CAD build for the part. Positions are in the model's coordinates, mm. Face numbers are marked on the shaded views. A direction names the side the tool comes from. Coordinates: 2 decimals unless noted, no trailing zeros. Loops run counter-clockwise (first coordinate to the right, second up) from the corner with the lowest first, then second, coordinate; pieces in that order, holes last.
1) Saw through at B-B, the plane x = 0. Write the cut outline in (y, z).
2) Saw through at D-D, the plane x = -11.5. Write the cut outline in (y, z).
3) Saw through at C-C, the plane z = -4.5. Write the cut outline in (x, y), and give its area (3 significant figures).
4) Pin check, flat tips, straight feed: pin 1 Ø15.5 at (x, z) = (-24, 0) entering from +Y; pin 2 Ø6.5 at (y, z) = (36, -13.5) entering from +X; pin 3 Ø4 at (x, z) = (-14.5, -19.5) entering from +Y. Stop position of each tip, or through.
5) Which spindle directions (+Z, -Z, +X, -X, +Y, -Y) get a long thin tool onto all of the face, cutting with end or side? Do the marked faces 1, 2, 3, 4 and 5. Say none if no direction does.
6) Wall check: line 1 along X through (y, z) = (5, 0); line 2 along X through (y, z) = (60, -19); line 3 along Y through (x, z) = (0, -14). Give the ranges that are in metal, low to high.
7) Two-plate mould, pull along X, no slides. Class the marked faces 6, 7 and 8: +X half, -X half, draft (parallel to the pull), parting line (faces both ways), or undercut.
8) Saw through at A-A, the plane z = -19. Write the cut outline in (x, y).
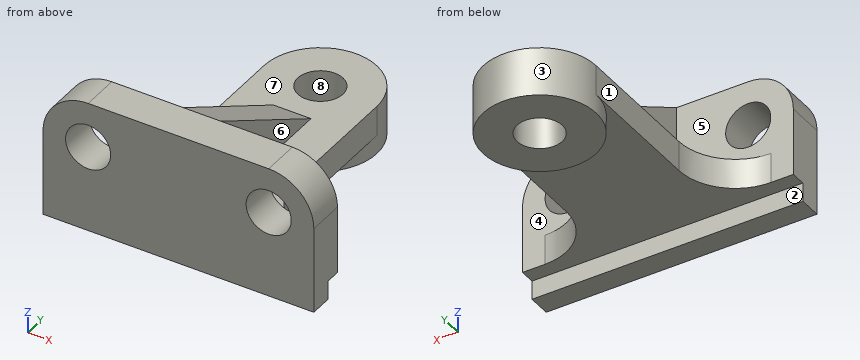
```python
from build123d import *

# Parameters (mm, degrees)
BASE_PLATE_SKETCH_R       = 6
BASE_PLATE_DEPTH          = 10
REAR_GROOVE_SKETCH_W      = 5
REAR_GROOVE_SKETCH_H      = 4
REAR_GROOVE_4X5_DEPTH     = 77.243032469
UPRIGHT_SKETCH_W          = 30
UPRIGHT_SKETCH_H          = 50
UPRIGHT_DEPTH             = 8
HUB_BOSS_SKETCH_R         = 15
HUB_BOSS_SKETCH_R_2       = 6
HUB_BOSS_DEPTH            = 13
SHAFT_START               = -13
SHAFT_BORE_SKETCH_R       = 6
SHAFT_BORE_DEPTH          = 13
UPRIGHT_BASE_FILLET_R15_R = 15
SUPPORT_RIB_REACH         = 88.313
SUPPORT_RIB_SKETCH_WALL_W = 218.626765016
SUPPORT_RIB_SKETCH_WALL_H = 10


with BuildPart() as part:
    # Base Plate Sketch → Base Plate (new body)
    with BuildSketch(Plane(origin=(0, 0, 0), x_dir=(1, 0, 0), z_dir=(0, 1, 0))):
        with BuildLine():
            Line((-36, 23), (-36, 0))
            ThreePointArc((-36, 0), (-32.485281374, -8.485281374), (-24, -12))
            Line((-24, -12), (24, -12))
            ThreePointArc((24, -12), (32.485281374, -8.485281374), (36, 0))
            Line((36, 0), (36, 23))
            Line((36, 23), (-36, 23))
        make_face()
        with Locations(Location((-24, 0, 0), (0, 0, 270))):
            Circle(BASE_PLATE_SKETCH_R, mode=Mode.SUBTRACT)
        with Locations(Location((24, 0, 0), (0, 0, 90))):
            Circle(BASE_PLATE_SKETCH_R, mode=Mode.SUBTRACT)
    extrude(amount=BASE_PLATE_DEPTH)

    # Rear Groove Sketch → Rear Groove 4x5 (cut, through all)
    with BuildSketch(Plane(origin=(36, 0, 0), x_dir=(0, 0, -1), z_dir=(1, 0, 0))):
        with Locations((20.5, 8)):
            Rectangle(REAR_GROOVE_SKETCH_W, REAR_GROOVE_SKETCH_H)
    extrude(amount=-REAR_GROOVE_4X5_DEPTH, mode=Mode.SUBTRACT)

    # Upright Sketch → Upright (add)
    with BuildSketch(Plane.XY.offset(-18)):
        with Locations((0, 35)):
            Rectangle(UPRIGHT_SKETCH_W, UPRIGHT_SKETCH_H)
    extrude(amount=UPRIGHT_DEPTH)

    # Hub Boss Sketch → Hub Boss (add)
    with BuildSketch(Plane.XY.offset(-10)):
        with Locations((0, 60)):
            Circle(HUB_BOSS_SKETCH_R)
        with Locations((0, 60)):
            Circle(HUB_BOSS_SKETCH_R_2, mode=Mode.SUBTRACT)
    extrude(amount=-HUB_BOSS_DEPTH)

    # Shaft Bore Sketch → Shaft Bore (cut)
    with BuildSketch(Plane(origin=(0, 0, -23), x_dir=(-1, 0, 0), z_dir=(0, 0, -1)).offset(SHAFT_START)):
        with Locations(Location((0, 60, 0), (0, 0, 180))):
            Circle(SHAFT_BORE_SKETCH_R)
    extrude(amount=SHAFT_BORE_DEPTH, mode=Mode.SUBTRACT)

    # Upright Base Fillet R15
    upright_base_fillet_r15_edges = [part.edges().sort_by_distance(p)[0] for p in [
        (-15, 10, -14),
        (15, 10, -14),
    ]]
    fillet(upright_base_fillet_r15_edges, radius=UPRIGHT_BASE_FILLET_R15_R)

    # Support Rib Sketch wall → Support Rib (add, up to next)
    with BuildSketch(Plane(origin=(0, 29.052558884, 1), x_dir=(0, 0.866025403787, -0.499999999995), z_dir=(0, 0.499999999995, 0.866025403787)), mode=Mode.PRIVATE) as support_rib_sk1:
        Rectangle(SUPPORT_RIB_SKETCH_WALL_W, SUPPORT_RIB_SKETCH_WALL_H)
    support_rib_tool1 = extrude(support_rib_sk1.sketch, amount=-SUPPORT_RIB_REACH, mode=Mode.PRIVATE) - part.part
    add(support_rib_tool1.solids().sort_by_distance((0, 29.052558884, 1))[0])


solid = part.part
```
Data:
1. outline: (0, -23) - (6, -23) - (6, -18) - (45, -18) - (45, -23) - (54, -23) - (54, -10) - (48.11, -10) - (10, 12) - (0, 12) - close; (66, -23) - (75, -23) - (75, -10) - (66, -10) - close
2. outline: (0, -23) - (6, -23) - (6, -18) - (50.37, -18) - (50.37, -23) - (69.63, -23) - (69.63, -10) - (10, -10) - (10, 12) - (0, 12) - close
3. outline: (-36, 0) - (-27.97, 0) - (-27.97, 10) - (-36, 10) - close; (-20.03, 0) - (20.03, 0) - (20.03, 10) - (5, 10) - (5, 38.58) - (-5, 38.58) - (-5, 10) - (-20.03, 10) - close; (27.97, 0) - (36, 0) - (36, 10) - (27.97, 10) - close
3. area: 847 mm2
4. pin 1: stops at y = 10
4. pin 2: stops at x = 15
4. pin 3: stops at y = 68.29
5. face 1: +Z, -Z, -X, +Y
5. face 2: -Z, +X, -X
5. face 3: -Z
5. face 4: +Z, +X, +Y
5. face 5: +Z, -X, +Y
6. line 1: x = -36 to -30, -18 to 18, 30 to 36
6. line 2: x = -15 to -6, 6 to 15
6. line 3: y = 0 to 54, 66 to 75
7. face 6: +X half
7. face 7: draft
7. face 8: undercut
8. outline: (-36, 0) - (36, 0) - (36, 6) - (-36, 6) - close; circle Ø30 at (0, 60); hole circle Ø12 at (0, 60)
